Verification items for the finished model (mm, model axes). A direction names the side the tool comes from. Round coordinates to 2 decimals unless told otherwise and drop trailing zeros. Order: outer loops, then holes, each group sorted by start corner. A loop starts at its lowest first (then second) coordinate and runs counter-clockwise, first axis right, second up. Notation, with made-up numbers: M -12,27 L 7,27 A18 cw 7,50 Z; hole C 77,-4.5 d6. An arc over 180 degrees is marked long. Answer as a JSON object with one key per item and string values. Group by question number.
```python
from build123d import *
from build123d.topology import SkipClean

# Parameters (mm, degrees)
SKETCH1_R               = 3.4
BOSS_EXTRUDE1_DEPTH     = 6
CHAMFER1_SIZE           = 1
SKETCH2_W               = 6
SKETCH2_H               = 20
BOSS_EXTRUDE2_DEPTH     = 30
CUT_EXTRUDE1_DEPTH      = 60.73483071
CUT_EXTRUDE1_DEPTH_BACK = 60.73483071
SKETCH3_R               = 2.75
SKETCH4_R               = 10
SKETCH4_R_2             = 2.75
BOSS_EXTRUDE3_DEPTH     = 1
CHAMFER2_SIZE           = 0.5
FILLET1_R               = 1
SKETCH5_W               = 20
SKETCH5_H               = 20
SKETCH5_R               = 3.4
BOSS_EXTRUDE4_DEPTH     = 5
CUT_EXTRUDE2_DEPTH      = 61.508263976
CUT_EXTRUDE2_DEPTH_BACK = 3
SKETCH7_R               = 6.95
SKETCH7_R_2             = 2.75
BOSS_EXTRUDE5_DEPTH     = 9.8
CHAMFER4_SIZE           = 0.5


with BuildPart() as part:
    # Sketch1 → Boss-Extrude1 (new body)
    with BuildSketch(Plane.XY):
        with BuildLine():
            Line((-26, 12.5), (26, 12.5))
            ThreePointArc((26, 12.5), (28.828427125, 11.328427125), (30, 8.5))
            Line((30, 8.5), (30, -8.5))
            ThreePointArc((30, -8.5), (28.828427125, -11.328427125), (26, -12.5))
            Line((26, -12.5), (-26, -12.5))
            ThreePointArc((-26, -12.5), (-28.828427125, -11.328427125), (-30, -8.5))
            Line((-30, -8.5), (-30, 8.5))
            ThreePointArc((-30, 8.5), (-28.828427125, 11.328427125), (-26, 12.5))
        make_face()
        Circle(SKETCH1_R, mode=Mode.SUBTRACT)
        with BuildLine():
            Line((-20.5, 5), (-20.5, -5))
            ThreePointArc((-20.5, -5), (-22.5, -7), (-24.5, -5))
            Line((-24.5, -5), (-24.5, 5))
            ThreePointArc((-24.5, 5), (-22.5, 7), (-20.5, 5))
        make_face(mode=Mode.SUBTRACT)
        with BuildLine():
            Line((20.5, 5), (20.5, -5))
            ThreePointArc((20.5, -5), (22.5, -7), (24.5, -5))
            Line((24.5, -5), (24.5, 5))
            ThreePointArc((24.5, 5), (22.5, 7), (20.5, 5))
        make_face(mode=Mode.SUBTRACT)
    extrude(amount=BOSS_EXTRUDE1_DEPTH)

    # Chamfer1
    chamfer1_edges = [part.edges().sort_by_distance(p)[0] for p in [
        (-3.4, 0, 0),
    ]]
    chamfer(chamfer1_edges, length=CHAMFER1_SIZE)

    # Sketch2 → Boss-Extrude2 (add)
    with BuildSketch(Plane.XY.offset(6)):
        with Locations((-13, 0)):
            Rectangle(SKETCH2_W, SKETCH2_H)
    extrude(amount=BOSS_EXTRUDE2_DEPTH)

    # Sketch3 → Cut-Extrude1 (cut, two sides: drawn at the far end of the back side and taken through both)
    with BuildSketch(Plane.ZY.offset(16).offset(-CUT_EXTRUDE1_DEPTH_BACK)):
        with Locations(Location((26, 0, 0), (0, 0, 270))):
            Circle(SKETCH3_R)
        with BuildLine():
            Line((26, 10), (26.394492089, 15.308450708))
            Line((26.394492089, 15.308450708), (43.333609146, 9.271325943))
            Line((43.333609146, 9.271325943), (37.706774414, -17.690590479))
            Line((37.706774414, -17.690590479), (26, -10))
            ThreePointArc((26, -10), (36, 0), (26, 10))
        make_face()
    extrude(amount=CUT_EXTRUDE1_DEPTH + CUT_EXTRUDE1_DEPTH_BACK, mode=Mode.SUBTRACT)

    # Sketch4 → Boss-Extrude3 (add, symmetric)
    with BuildSketch(Plane.ZY.offset(16)):
        with Locations(Location((26, 0, 0), (0, 0, 270))):
            Circle(SKETCH4_R)
        with Locations(Location((26, 0, 0), (0, 0, 270))):
            Circle(SKETCH4_R_2, mode=Mode.SUBTRACT)
    extrude(amount=BOSS_EXTRUDE3_DEPTH, both=True)

    # Chamfer2
    chamfer2_edges = [part.edges().sort_by_distance(p)[0] for p in [
        (-17, 10, 26),
    ]]
    chamfer(chamfer2_edges, length=CHAMFER2_SIZE)

    # Fillet1
    fillet1_edges = [part.edges().sort_by_distance(p)[0] for p in [
        (28.828427125, -11.328427125, 6),
        (30, 0, 6),
        (28.828427125, 11.328427125, 6),
        (0, 12.5, 6),
        (-28.828427125, 11.328427125, 6),
        (-30, 0, 6),
        (-28.828427125, -11.328427125, 6),
        (0, -12.5, 6),
    ]]
    fillet(fillet1_edges, radius=FILLET1_R)

    # Sketch5 → Boss-Extrude4 (add)
    with BuildSketch(Plane.XY.offset(6)):
        Rectangle(SKETCH5_W, SKETCH5_H)
        Circle(SKETCH5_R, mode=Mode.SUBTRACT)
    extrude(amount=BOSS_EXTRUDE4_DEPTH)

    # Sketch6 → Cut-Extrude2 (cut, two sides: drawn at the far end of the back side and taken through both)
    with BuildSketch(Plane.ZY.offset(17).offset(-CUT_EXTRUDE2_DEPTH_BACK)):
        Polygon((28.369738511, 4.098496398), (23.635467258, 4.10150195), (21.265728747, 0.003005552), (23.630261489, -4.098496398), (28.364532742, -4.10150195), (30.734271253, -0.003005552), align=None)
    extrude(amount=CUT_EXTRUDE2_DEPTH + CUT_EXTRUDE2_DEPTH_BACK, mode=Mode.SUBTRACT)

    # Sketch7 → Boss-Extrude5 (add)
    with SkipClean():  # the faces are left unmerged after this step: merging them gives an invalid solid
        with BuildSketch(Plane(origin=(-10, 0, 0), x_dir=(0, 0, -1), z_dir=(1, 0, 0))):
            with Locations(Location((-26, 0, 0), (0, 0, 270))):
                Circle(SKETCH7_R)
            with Locations(Location((-26, 0, 0), (0, 0, 180))):
                Circle(SKETCH7_R_2, mode=Mode.SUBTRACT)
        extrude(amount=BOSS_EXTRUDE5_DEPTH)

    # Chamfer4
    chamfer4_edges = [part.edges().sort_by_distance(p)[0] for p in [
        (-0.2, 6.95, 26),
    ]]
    chamfer(chamfer4_edges, length=CHAMFER4_SIZE)


solid = part.part
```
Q1. Gauge pin test, flat ends, axial feed: pin 1 Ø8 at (x, z) = (-14, 21) entering from -Y; pin 2 Ø4 at (y, z) = (-1.5, 7.5) entering from +X; pin 3 Ø10 at (y, z) = (-9, 8) entering from +X; pin 4 Ø1 at (x, y) = (10, 1.5) entering from +Z. Record the tip position at first contact, or that the pin passes through.
Q2. Release check for a two-part mould opening along Z. For faces 1 (the face through (-10, 0, 18)), 2 (the face through (0, 6, 0)), 3 (the face through (22.5, -7, 3)) record: released by +Z, released by -Z, zero draft, split by the parting line, or undercut.
Q3. Cross-section at C-C, the plane y = 2. Give the number of separate pieces and of enclosed holes in the cut face, then the cut area to 3 significant figures.
Q4. Tool access check on faces 4 (the face through (-9, -10, 9)), 5 (the face through (-0.74, -3.32, 5.93)), 6 (the face through (22.5, 7, 3)), 7 (the face through (-14, 3, 26)), 8 (the face through (10, 0, 8)). Record the directions out of +Z, -Z, +X, -X, +Y, -Y that give a thin tool (end or side, any length) a straight path to the whole face; none if there is none.
Q5. Cross-section at A-A, the plane x = -9. Record the cut outline in (y, z), then the cut area to 3 significant figures.
Q6. Cross-section at B-B, the plane z = 10. Record the cut outline in (x, y).
Q7. Thickness scan on line 1 (Y direction, x = -5, z = 26); line 2 (Z direction, x = 18.5, y = -7); line 3 (X direction, y = 2.5, z = 4.5). Record the ranges inside material, lowest first. Write a range as from..to.
Conclusion:
{
 "1": {"pin 1": "y = -10", "pin 2": "x = 29.87", "pin 3": "x = 30", "pin 4": "z = 11"},
 "2": {"face 1": "undercut", "face 2": "released by -Z", "face 3": "zero draft"},
 "3": {"separate pieces": "5", "enclosed holes": "0", "area": "605 mm2"},
 "4": {"face 4": "+Z, +X, -X, -Y", "face 5": "-Z", "face 6": "+Z, -Z", "face 7": "-X", "face 8": "+Z, +X, +Y, -Y"},
 "5": {"outline": "M -12.5,0 L 12.5,0 L 12.5,5 A1 ccw 11.5,6 L 10,6 L 10,11 L -10,11 L -10,6 L -11.5,6 A1 ccw -12.5,5 Z; C 0,26 d13.9; hole C 0,26 d5.5", "area": "378 mm2"},
 "6": {"outline": "M -16,-10 L 10,-10 L 10,10 L -16,10 Z; hole C 0,0 d6.8"},
 "7": {"line 1": "-6.95..-2.75, 2.75..6.95", "line 2": "0..6", "line 3": "-30..-24.5, -20.5..-2.3, 2.3..20.5, 24.5..30"}
}
